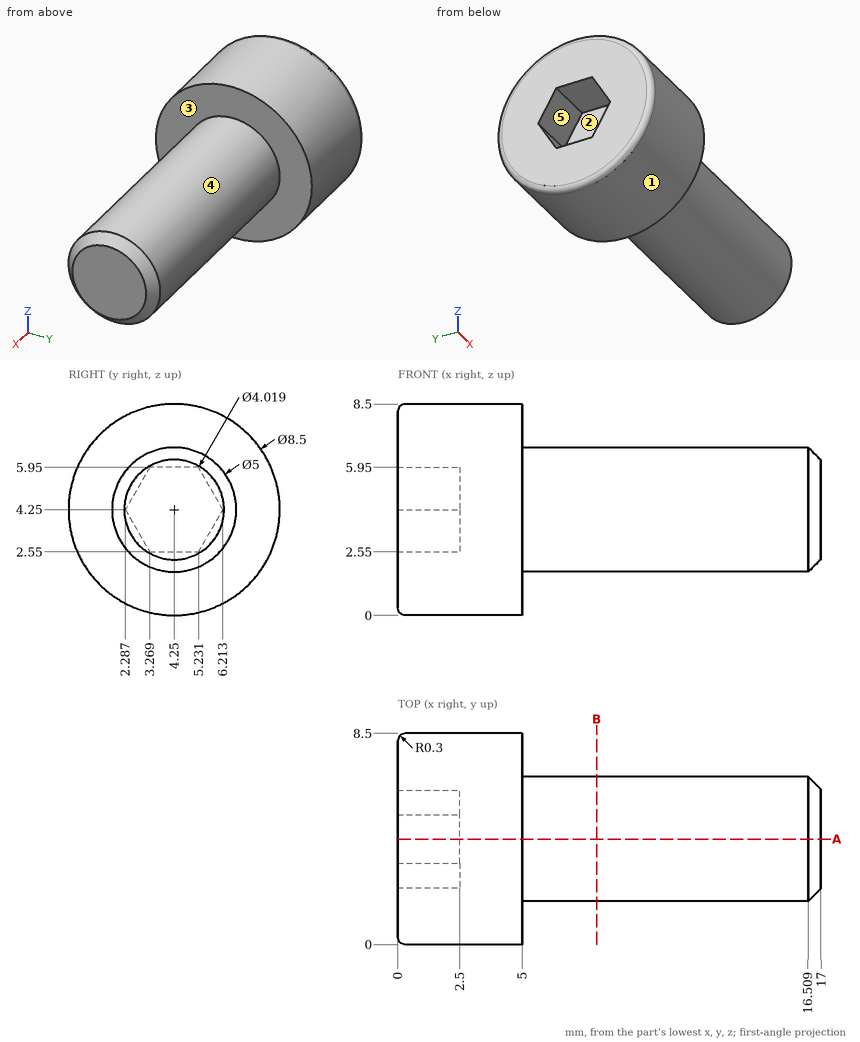
Could you check a few things on this drawing? It's one solid part, dimensions in mm from its lowest x, y, z. A direction names the side the tool comes from. Coordinates: 2 decimals unless noted, no trailing zeros. Write each loop counter-clockwise with the first axis right and the second up, starting at its lowest first coordinate (ties: lowest second). Pieces come first, ordered by that corner, then holes.
Q1. If we mould it in two halves opening along Y, with no side actions, what happens to the marked faces 3, 4 and 5? For each: +Y half, -Y half, draft (parallel to the pull), parting line (faces both ways), or undercut.
Results found:
face 3: draft
face 4: parting line
face 5: undercut
Q2. Imagine slicing it at A-A, the plane y = 4.25. List the corners of the cut face in (x, z) for me.
Results found:
outline: (0, 0.3) arc R0.3 ccw to (0.3, 0) - (5, 0) - (5, 1.75) - (16.51, 1.75) - (17, 2.24) - (17, 6.26) - (16.51, 6.75) - (5, 6.75) - (5, 8.5) - (0.3, 8.5) arc R0.3 ccw to (0, 8.2) - (0, 5.95) - (2.5, 5.95) - (2.5, 2.55) - (0, 2.55) - close
Q3. For P1, Ø3, axis at x = 14, y = 5, coming from the +Z side; P2, Ø0.6, axis at x = 1, y = 4.5, coming from the +Z side; P3, Ø4, axis at x = 8, z = 5.5, coming from the +Y side; P4, Ø3, axis at x = 3, y = 7.5, coming from the +Z side, each with a flat end and sliding along its axis, tell me the tip position at first contact or that it passes through.
Results found:
P1: stops at z = 6.75
P2: stops at z = 8.5
P3: stops at y = 6.75
P4: stops at z = 8.12
Q4. Which directions (+Z, -Z, +X, -X, +Y, -Y) give clear straight access to the entire face, cutting with the end or side of a thin tool? Please do the marked faces 1 and 2.
Results found:
face 1: +X, -X
face 2: -X
Q5. Imagine slicing it at B-B, the plane x = 8. List the corners of the cut face in (y, z) for me.
Results found:
outline: circle Ø5 at (4.25, 4.25)
Q6. Please list where these lines run through material, in increasing order: L1, parallel to X at y = 2.25, z = 7.25; L2, parallel to X at y = 4.5, z = 5.5; L3, parallel to Y at x = 13.5, z = 4.75.
Results found:
L1: x = 0 to 5
L2: x = 2.5 to 17
L3: y = 1.8 to 6.7
